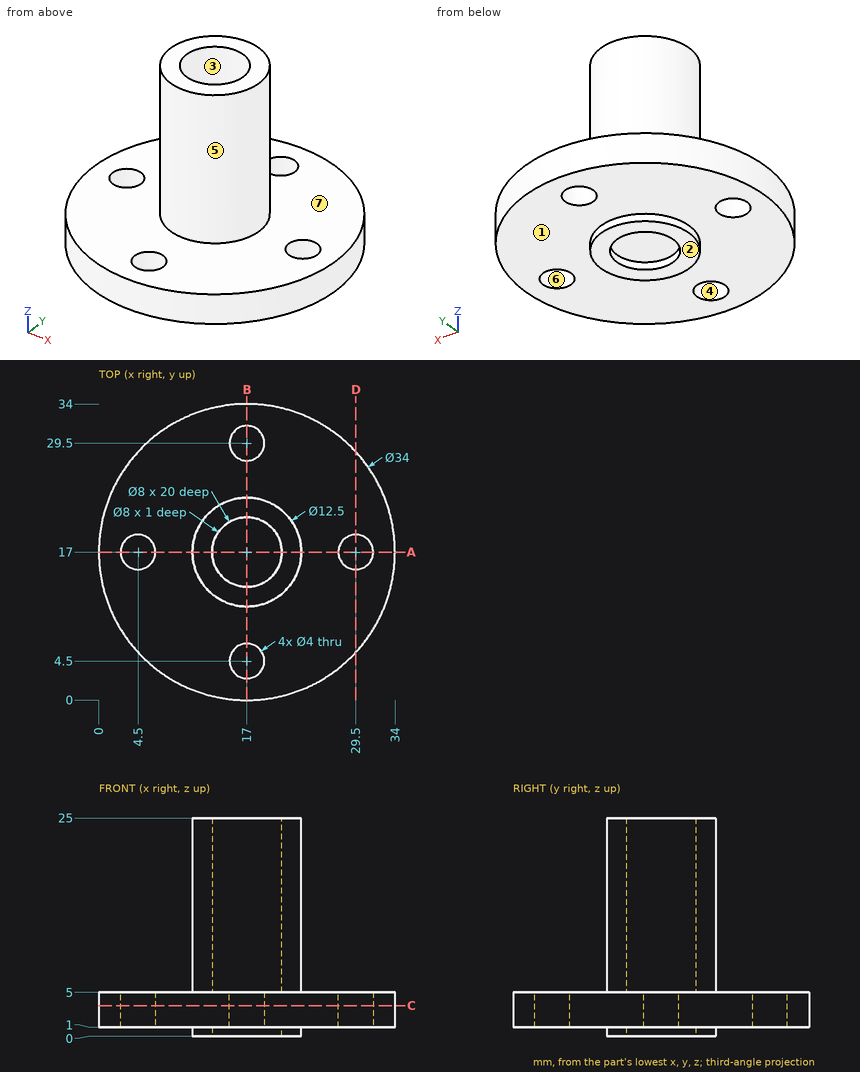
Geometry check sheet. Reference: drawing and pictorial views, mm from the part's lowest x, y, z. A direction names the side the tool comes from. Give positions to 0.01 mm unless a question says otherwise; leave off trailing zeros. Write each loop counter-clockwise with the first axis right and the second up, starting at its lowest first coordinate (ties: lowest second). Pieces come first, ordered by that corner, then holes.
Item 1: Draft check along Y on the marked faces 4, 5, 6 and 7. Enter one of: released by +Y, released by -Y, zero draft, split by the parting line, or undercut.
Item 2: Cross-section at A-A (y = 17). Enter the section's corners in (x, z), and give its area (4 significant figures).
Item 3: Cross-section at C-C (z = 3.5). Enter the section's corners in (x, y), and give its area (3 significant figures).
Item 4: Access from +Z, -Z, +X, -X, +Y, -Y to the whole of each face (thin tool, end or side, straight path). Record for the marked faces 1, 2 and 3.
Item 5: Cross-section at D-D (x = 29.5). Enter the section's corners in (y, z).
Item 6: Gauge pin test, flat ends, axial feed: pin 1 (3 mm diameter, centred on x = 18, z = 16, fed in from -Y); pin 2 (4 mm diameter, centred on x = 7, z = 10.5, fed in from -Y); pin 3 (2 mm diameter, centred on x = 20.5, y = 20, fed in from -Z); pin 4 (5 mm diameter, centred on x = 17, y = 17, fed in from +Z). Record the tip position at first contact, or that the pin passes through.
Item 7: Scan lines: L1, parallel to X at y = 17, z = 0.45; L2, parallel to Z at x = 9, y = 31. Record each from-to range of solid material in increasing order.
Report:
1. face 4: undercut
1. face 5: split by the parting line
1. face 6: undercut
1. face 7: zero draft
2. outline: (0, 1) - (2.5, 1) - (2.5, 5) - (0, 5) - close; (6.5, 1) - (10.75, 1) - (10.75, 0) - (13, 0) - (13, 1) - (21, 1) - (21, 0) - (23.25, 0) - (23.25, 1) - (27.5, 1) - (27.5, 5) - (23.25, 5) - (23.25, 25) - (21, 25) - (21, 5) - (13, 5) - (13, 25) - (10.75, 25) - (10.75, 5) - (6.5, 5) - close; (31.5, 1) - (34, 1) - (34, 5) - (31.5, 5) - close
2. area: 198.5 mm2
3. outline: circle Ø34 at (17, 17); hole circle Ø4 at (4.5, 17); hole circle Ø4 at (17, 4.5); hole circle Ø4 at (17, 29.5); hole circle Ø4 at (29.5, 17)
3. area: 858 mm2
4. face 1: -Z
4. face 2: -Z, +X, -X, +Y, -Y
4. face 3: +Z
5. outline: (5.48, 1) - (15, 1) - (15, 5) - (5.48, 5) - close; (19, 1) - (28.52, 1) - (28.52, 5) - (19, 5) - close
6. pin 1: stops at y = 10.75
6. pin 2: passes through
6. pin 3: stops at z = 0
6. pin 4: stops at z = 5
7. L1: x = 10.75 to 13, 21 to 23.25
7. L2: z = 1 to 5
